CAD build for the part. Positions are in the model's coordinates, mm. A direction names the side the tool comes from. Give positions to 0.01 mm unless a question says otherwise; leave off trailing zeros. Loops run counter-clockwise (first coordinate to the right, second up) from the corner with the lowest first, then second, coordinate; pieces in that order, holes last.
Item 1: Mould opens along X. For faces 1 (the flat face through (592, 0, 148)), 2 (the flat face through (592, -493, 2)), 3 (the flat face through (0, -507, 148)) say: released by +X, released by -X, zero draft, split by the parting line, or undercut.
Item 2: Drop flat-ended pins along their axis: P1, Ø3, axis at x = 60.5, y = -907.5, coming from the +Z side; P2, Ø6, axis at x = 203, y = -299.5, coming from the +Z side. Give the stop position or say it passes through.
Item 3: Probe probe 1 along X at (y, z) = (-492.5, 16.5); probe 2 along Y at (x, z) = (60, 1.5); probe 3 along Z at (x, y) = (421.5, -104). List the from-to ranges inside material, lowest first.
Item 4: Saw through at C-C on z = 233. Give the cut face in (x, y), plus the area to 3 significant figures.
Item 5: Which spindle directions (+Z, -Z, +X, -X, +Y, -Y) get a long thin tool onto all of the face, cutting with end or side? Do faces 4 (the flat face through (592, -493, 32)), 5 (the flat face through (1200, -507, 148)), 6 (the flat face through (592, -493, 34)). Say none if no direction does.
Item 6: Saw through at B-B on y = -774.5. Give the cut face in (x, z), plus the area to 3 significant figures.
Item 7: Saw through at A-A on x = 621. Give the cut face in (y, z), plus the area to 3 significant figures.
from build123d import *

# Parameters (mm, degrees)
SKETCH_1_W                     = 1200
SKETCH_1_H                     = 1000
EXTRUDE_1_DEPTH                = 300
SHELL_1_T                      = -2
SKETCH_2_R                     = 7
CUT_EXTRUDE_1_DEPTH            = 1591.221368238
PATTERN_LINEAR_1_COUNT         = 3
PATTERN_LINEAR_1_PITCH         = 388
PATTERN_LINEAR_2_COUNT         = 3
PATTERN_LINEAR_2_PITCH         = 538
SKETCH_3_W                     = 1200
SKETCH_3_H                     = 1000
SKETCH_3_W_2                   = 1160
SKETCH_3_H_2                   = 960
EXTRUDE_2_DEPTH                = 2
SKETCH_4_W                     = 1164
SKETCH_4_H                     = 964
SKETCH_4_W_2                   = 1160
SKETCH_4_H_2                   = 960
EXTRUDE_3_DEPTH                = 20
EXTRUDE_START                  = 30
SKETCH_5_W                     = 1120
SKETCH_5_H                     = 940
EXTRUDE_4_DEPTH                = 2
SKETCH_6_W                     = 1120
SKETCH_6_H                     = 940
SKETCH_6_W_2                   = 1116
SKETCH_6_H_2                   = 936
EXTRUDE_5_DEPTH                = 22
SKETCH_8_R                     = 6
EXTRUDE_6_DEPTH                = 50
FILLET_1_R                     = 1
EXTRUDE_7_DEPTH                = 10
PATTERN_LINEAR_4_COUNT         = 2
PATTERN_LINEAR_4_PITCH         = 1080
PATTERN_LINEAR_4_COUNT_DIR2    = 2
PATTERN_LINEAR_4_PITCH_DIR2    = 820
FILLET_1_OF_PATTERN_LINEAR_4_R = 1


with BuildPart() as part:
    # Sketch 1 → Extrude 1 (new body)
    with BuildSketch(Plane.XY):
        with Locations((600, -500)):
            Rectangle(SKETCH_1_W, SKETCH_1_H)
    extrude(amount=EXTRUDE_1_DEPTH)

    # Shell 1
    shell_1_openings = [part.faces().sort_by_distance(p)[0] for p in [
        (600, -500, 300),
    ]]
    offset(amount=SHELL_1_T, openings=shell_1_openings, kind=Kind.INTERSECTION)

    # Sketch 2 → Cut-Extrude 1 (cut, through all)
    with BuildSketch(Plane.XY.offset(2)):
        with Locations((60, -62)):
            Circle(SKETCH_2_R)
    cut_extrude_1 = extrude(amount=-CUT_EXTRUDE_1_DEPTH, mode=Mode.SUBTRACT)

    # Pattern Linear 1: Cut-Extrude 1 ×3
    with Locations(*[(0, -i * PATTERN_LINEAR_1_PITCH, 0) for i in range(1, PATTERN_LINEAR_1_COUNT)]):
        add(cut_extrude_1, mode=Mode.SUBTRACT)

    # Pattern Linear 2: Cut-Extrude 1 ×3
    with Locations(*[(i * PATTERN_LINEAR_2_PITCH, 0, 0) for i in range(1, PATTERN_LINEAR_2_COUNT)]):
        add(cut_extrude_1, mode=Mode.SUBTRACT)

    # Sketch 3 → Extrude 2 (add)
    with BuildSketch(Plane.XY.offset(300)):
        with Locations((600, -500)):
            Rectangle(SKETCH_3_W, SKETCH_3_H)
        with Locations((600, -500)):
            Rectangle(SKETCH_3_W_2, SKETCH_3_H_2, mode=Mode.SUBTRACT)
    extrude(amount=-EXTRUDE_2_DEPTH)

    # Sketch 4 → Extrude 3 (add)
    with BuildSketch(Plane.XY.offset(300)):
        with Locations((600, -500)):
            Rectangle(SKETCH_4_W, SKETCH_4_H)
        with Locations((600, -500)):
            Rectangle(SKETCH_4_W_2, SKETCH_4_H_2, mode=Mode.SUBTRACT)
    extrude(amount=-EXTRUDE_3_DEPTH)



with BuildPart() as body_2:
    # Sketch 5 → Extrude 4 (new body)
    with BuildSketch(Plane.XY.offset(2).offset(EXTRUDE_START)):
        with Locations((600, -500)):
            Rectangle(SKETCH_5_W, SKETCH_5_H)
    extrude(amount=EXTRUDE_4_DEPTH)

    # Sketch 6 → Extrude 5 (add)
    with BuildSketch(Plane.XY.offset(34)):
        with Locations((600, -500)):
            Rectangle(SKETCH_6_W, SKETCH_6_H)
        with Locations((600, -500)):
            Rectangle(SKETCH_6_W_2, SKETCH_6_H_2, mode=Mode.SUBTRACT)
    extrude(amount=-EXTRUDE_5_DEPTH)


with BuildPart() as part_1:
    add(part.part)

    add(body_2.part)  # Extrude 6 merges body 2
    # Sketch 8 → Extrude 6 (add)
    with BuildSketch(Plane.XY.offset(2)):
        with Locations((60, -90)):
            Circle(SKETCH_8_R)
    extrude_6 = extrude(amount=EXTRUDE_6_DEPTH)

    # Fillet 1
    fillet_1_edges = [part_1.edges().sort_by_distance(p)[0] for p in [
        (54, -90, 52),
    ]]
    fillet(fillet_1_edges, radius=FILLET_1_R)

    # Sketch 9 → Extrude 7 (add)
    with BuildSketch(Plane.XY.offset(34)):
        Polygon((66, -79.607695155), (54, -79.607695155), (48, -90), (54, -100.392304845), (66, -100.392304845), (72, -90), align=None)
    extrude_7 = extrude(amount=EXTRUDE_7_DEPTH)

    # Pattern Linear 4: Extrude 6, Extrude 7 2 × 2
    with Locations(*[(i * PATTERN_LINEAR_4_PITCH, -j * PATTERN_LINEAR_4_PITCH_DIR2, 0) for i in range(PATTERN_LINEAR_4_COUNT) for j in range(PATTERN_LINEAR_4_COUNT_DIR2) if (i, j) != (0, 0)]):
        add(extrude_6)
        add(extrude_7)

    # Fillet 1 of Pattern Linear 4
    fillet_1_of_pattern_linear_4_edges = [part_1.edges().sort_by_distance(p)[0] for p in [
        (54, -910, 52),
        (1134, -90, 52),
        (1134, -910, 52),
    ]]
    fillet(fillet_1_of_pattern_linear_4_edges, radius=FILLET_1_OF_PATTERN_LINEAR_4_R)


solid = part_1.part
Results below:
1. face 1: zero draft
1. face 2: undercut
1. face 3: released by -X
2. P1: stops at z = 52
2. P2: stops at z = 34
3. probe 1: x = 0 to 2, 40 to 42, 1158 to 1160, 1198 to 1200
3. probe 2: y = -1000 to -845, -831 to -457, -443 to -69, -55 to 0
3. probe 3: z = 0 to 2, 32 to 34
4. outline: (0, -1000) - (1200, -1000) - (1200, 0) - (0, 0) - close; hole (2, -998) - (1198, -998) - (1198, -2) - (2, -2) - close
4. area: 8,780 mm2
5. face 4: none
5. face 5: +Z, -Z, +X, +Y, -Y
5. face 6: +Z
6. outline: (0, 0) - (1200, 0) - (1200, 300) - (1180, 300) - (1180, 280) - (1182, 280) - (1182, 298) - (1198, 298) - (1198, 2) - (2, 2) - (2, 298) - (18, 298) - (18, 280) - (20, 280) - (20, 300) - (0, 300) - close; (40, 12) - (42, 12) - (42, 32) - (1158, 32) - (1158, 12) - (1160, 12) - (1160, 34) - (40, 34) - close
6. area: 6,060 mm2
7. outline: (-1000, 0) - (0, 0) - (0, 300) - (-20, 300) - (-20, 280) - (-18, 280) - (-18, 298) - (-2, 298) - (-2, 2) - (-998, 2) - (-998, 298) - (-982, 298) - (-982, 280) - (-980, 280) - (-980, 300) - (-1000, 300) - close; (-970, 12) - (-968, 12) - (-968, 32) - (-32, 32) - (-32, 12) - (-30, 12) - (-30, 34) - (-970, 34) - close
7. area: 5,300 mm2
